from build123d import *

# Parameters (mm, degrees)
EXTRUDE_1_DEPTH       = 1.5
HOLE_WIZARD_6_0_6_1_D = 6
FILLET_1_R            = 3


with BuildPart() as part:
    # 草图1 → 凸台-拉伸1 (new body)
    with BuildSketch(Plane.XY):
        Polygon((-12.5, 0), (12.5, 0), (12.5, -29), (0, -50.650635095), (-12.5, -29), align=None)
    extrude(amount=EXTRUDE_1_DEPTH)

    # Ø6.0 (6) 直径孔1 (through all)
    with Locations(Plane.XY.offset(1.5)):
        with Locations((-7.5, -6), (7.5, -6)):
            Hole(HOLE_WIZARD_6_0_6_1_D / 2)

    # 圆角1
    fillet_1_edges = [part.edges().sort_by_distance(p)[0] for p in [
        (-12.5, 0, 0.75),
        (12.5, 0, 0.75),
    ]]
    fillet(fillet_1_edges, radius=FILLET_1_R)


solid = part.part
Geometry: final body of the model. Coordinates: model frame, mm. Give positions to 0.01 mm unless a question says otherwise; leave off trailing zeros. Loops run counter-clockwise (first coordinate to the right, second up) from the corner with the lowest first, then second, coordinate; pieces in that order, holes last. Notation, with made-up numbers: (-38, 78) -> (-4, 78) arc R21 ccw to (-4, 94) -> close; hole circle Ø4 at (54, -13.5). An arc over 180 degrees is marked (long way). Put each result on its own line as item: value.
1. Cut plane A-A (y = -6). Return the cut outline in (x, z).
Taken from the geometry:
outline: (-12.5, 0) -> (-10.5, 0) -> (-10.5, 1.5) -> (-12.5, 1.5) -> close; (-4.5, 0) -> (4.5, 0) -> (4.5, 1.5) -> (-4.5, 1.5) -> close; (10.5, 0) -> (12.5, 0) -> (12.5, 1.5) -> (10.5, 1.5) -> close
2. Ray query, line 1 along X through (y, z) = (-3.5, 0.2); line 2 along Y through (x, z) = (-7.5, 0.6); line 3 along X through (y, z) = (-41, 1.15). Return the intervals inside material, ascending. Write a range as [from, to].
Taken from the geometry:
line 1: x = [-12.5, -9.16], [-5.84, 5.84], [9.16, 12.5]
line 2: y = [-37.66, -9], [-3, 0]
line 3: x = [-5.57, 5.57]
3. Cut plane B-B (x = 7.75). Return the cut outline in (y, z).
Taken from the geometry:
outline: (-37.23, 0) -> (-8.99, 0) -> (-8.99, 1.5) -> (-37.23, 1.5) -> close; (-3.01, 0) -> (0, 0) -> (0, 1.5) -> (-3.01, 1.5) -> close
4. Cut plane D-D (x = -7.5). Return the cut outline in (y, z), plus the area to 3 significant figures.
Taken from the geometry:
outline: (-37.66, 0) -> (-9, 0) -> (-9, 1.5) -> (-37.66, 1.5) -> close; (-3, 0) -> (0, 0) -> (0, 1.5) -> (-3, 1.5) -> close
area: 47.5 mm2
5. Pull-direction query (X, two-part tool) for faces 1 (the cylindrical face through (5.89, -3.47, 0.74)), 2 (the cylindrical face through (-11.6, -0.86, 0.76)), 3 (the flat face through (0, -19, 0)); classes: released by +X, released by -X, zero draft, split by the parting line, or undercut.
Taken from the geometry:
face 1: undercut
face 2: released by -X
face 3: zero draft
6. Cut plane C-C (z = 0.8). Return the cut outline in (x, y).
Taken from the geometry:
outline: (-12.5, -29) -> (0, -50.65) -> (12.5, -29) -> (12.5, -3) arc R3 ccw to (9.5, 0) -> (-9.5, 0) arc R3 ccw to (-12.5, -3) -> close; hole circle Ø6 at (-7.5, -6); hole circle Ø6 at (7.5, -6)
